Could you check a few things on this model? Use its own coordinates, in mm. Face numbers are marked on the shaded views. Coordinates: 2 decimals unless noted, no trailing zeros. Loops run counter-clockwise (first coordinate to the right, second up) from the corner with the lowest first, then second, coordinate; pieces in that order, holes last. Notation, with made-up numbers: (86.25, 33) - (123.25, 33) arc R18 ccw to (123.25, 43) - close; hole circle Ø6 at (45.25, -30.5). An arc over 180 degrees is marked (long way). One line per question, with ' | ' between items. Start each with the question number.
1. I want a section at A-A, the plane x = -6.5. Write out the boundary of the cut face in (y, z), then the cut area to 3 significant figures.
2. We'd pull the mould along X, two halves only. Please class the marked faces 1, 2 and 3: pulls with the +X half, pulls with the -X half, needs draft (parallel to the pull), parting line crosses it, or undercut.
3. Please list where these lines run through material, in increasing order: L1, parallel to X at y = 19.5, z = 27; L2, parallel to X at y = -28, z = 2; L3, parallel to Y at x = 14.4, z = 0. Write a range as [from, to].
4. I'm going to push flat-ended pins straight in: P1, Ø6, axis at x = 6.5, z = 19, coming from the -Y side; P2, Ø3, axis at x = -11, z = 14.5, coming from the +Y side; P3, Ø4, axis at x = -9.5, y = -29, coming from the +Z side; P4, Ø10, axis at y = -10.5, z = -18, coming from the -X side. Where does each tip first touch, or does it pass through?
5. I want a section at B-B, the plane x = -12.5. Write out the boundary of the cut face in (y, z), then the cut area to 3 significant figures.
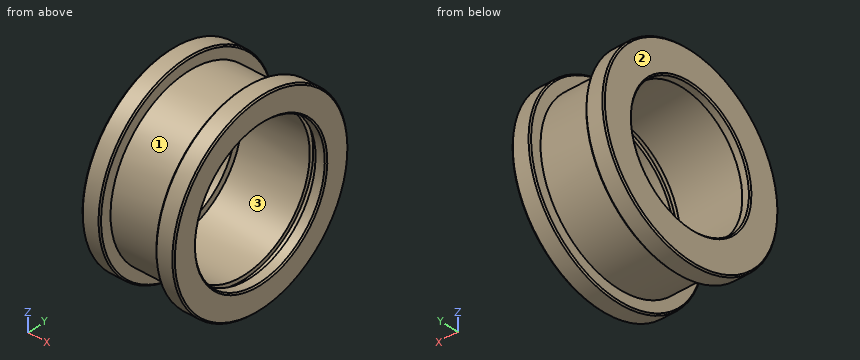
from build123d import *

# Parameters (mm, degrees)
SKETCH_2_R          = 27.5
CUT_EXTRUDE_1_DEPTH = 32
SKETCH_4_R          = 25
CUT_EXTRUDE_2_DEPTH = 30
CHAMFER_1_SIZE      = 0.5
SKETCH_5_W          = 2.2
SKETCH_5_H          = 1.5


with BuildPart() as part:
    # 草图1 → 旋转1 (revolve)
    with BuildSketch(Plane.XY, mode=Mode.PRIVATE) as revolve_1_sk:
        Polygon((-17.5, 0), (17.5, 0), (17.5, 37), (10.5, 37), (10.5, 32.5), (-10.5, 32.5), (-10.5, 37), (-17.5, 37), align=None)
    revolve(revolve_1_sk.sketch.rotate(Axis((-17.5, 0, 0), (1, 0, 0)), 90), axis=Axis((-17.5, 0, 0), (1, 0, 0)))

    # 草图2 → 切除-拉伸1 (cut)
    with BuildSketch(Plane(origin=(17.5, 0, 0), x_dir=(0, 0, -1), z_dir=(1, 0, 0))):
        Circle(SKETCH_2_R)
    extrude(amount=-CUT_EXTRUDE_1_DEPTH, mode=Mode.SUBTRACT)

    # 草图4 → 切除-拉伸2 (cut)
    with BuildSketch(Plane(origin=(-14.5, 0, 0), x_dir=(0, 0, -1), z_dir=(1, 0, 0))):
        Circle(SKETCH_4_R)
    extrude(amount=-CUT_EXTRUDE_2_DEPTH, mode=Mode.SUBTRACT)

    # 倒角1
    chamfer_1_edges = [part.edges().sort_by_distance(p)[0] for p in [
        (17.5, 0, 27.5),
        (-17.5, 0, 25),
        (-17.5, 0, -37),
        (-10.5, 0, -37),
        (10.5, 0, -37),
        (17.5, 0, -37),
    ]]
    chamfer(chamfer_1_edges, length=CHAMFER_1_SIZE)

    # 草图5 → 切除-旋转1 (revolve, cut)
    with BuildSketch(Plane(origin=(0, 0, 0), x_dir=(1, 0, 0), z_dir=(0, 1, 0))):
        with Locations((12.4, 28.25)):
            Rectangle(SKETCH_5_W, SKETCH_5_H)
    revolve(axis=Axis((0, 0, 0), (1, 0, 0)), mode=Mode.SUBTRACT)


solid = part.part
Results are:
1) outline: circle Ø65 at (0, 0); hole circle Ø55 at (0, 0) | area: 942 mm2
2) face 1: undercut | face 2: pulls with the -X half | face 3: needs draft
3) L1: x = [-17.5, -10.5], [10.5, 17.5] | L2: x = [-17.5, 11.3], [13.5, 17.5] | L3: y = [-37, -27.5], [27.5, 37]
4) P1: stops at y = -28.29 | P2: stops at y = 34.64 | P3: stops at z = 24.56 | P4: stops at x = -17.5
5) outline: circle Ø74 at (0, 0); hole circle Ø55 at (0, 0) | area: 1,930 mm2
